Part model, mm, in its own coordinate system. A direction names the side the tool comes from. Coordinates: 2 decimals unless noted, no trailing zeros. Order: outer loops, then holes, each group sorted by start corner. A loop starts at its lowest first (then second) coordinate and runs counter-clockwise, first axis right, second up. Notation, with made-up numbers: (71, -18) - (104, -18) arc R22 cw to (104, 21) - close; hole circle Ø6 at (-31.5, -4). An arc over 180 degrees is marked (long way). Use a Markdown table: item, result. Add a question column.
1) Tool access for faces 5 (the face through (-19.86, 0.54, 14.84)), 6 (the face through (-13.25, 13.79, 3.06)), 7 (the face through (19.963, -13.457, -0.104)): list every direction of +Z, -Z, +X, -X, +Y, -Y with a clear straight run to the whole face (end or side of a thin tool).
2) Saw through at A-A on x = 11.5. List the corners of the cut face in (y, z), then the cut area to 3 significant figures.
3) Two-plate mould, pull along Z, no slides. Class faces 1 (the face through (21.151, -7.35, -7.35)), 2 (the face through (19.46, 15.62, 3.47)), 3 (the face through (21.82, 9.05, -4.71)), 4 (the face through (22.498, 12, -4)): +Z half, -Z half, draft (parallel to the pull), parting line (faces both ways), or undercut.
4) Wall check: L1, parallel to Y at x = -17.5, z = 0; L2, parallel to Y at x = 18, z = 0; L3, parallel to Z at x = 20.5, y = 0.5. Give the ranges that are in metal, low to high. Write a range as [from, to].
5) Drop flat-ended pins along their axis: P1, Ø4, axis at x = -1, y = -4.5, coming from the -Z side (3 decimals); P2, Ø1.4, axis at y = 0, z = -14.25, coming from the +X side; P3, Ø1.5, axis at y = -4.5, z = 6, coming from the +X side. Give the stop position or say it passes through.
```python
from build123d import *

# Parameters (mm, degrees)
HOLE_WIZARD_M2_1_D     = 1.6
HOLE_WIZARD_M2_1_DEPTH = 5
HOLE_WIZARD_M2_1_TIP   = 0.480688495
HOLE_WIZARD_M2_2_D     = 1.6
HOLE_WIZARD_M2_2_DEPTH = 5.2
HOLE_WIZARD_M2_2_TIP   = 0.480688495
SKETCH_9_R             = 1.25
CUT_EXTRUDE_1_DEPTH    = 20


with BuildPart() as part:
    # 草图1 → 旋转1 (revolve)
    with BuildSketch(Plane.XY, mode=Mode.PRIVATE) as revolve_1_sk:
        Polygon((16.5, 16), (13.035898385, 14), (-13.035898385, 14), (-16.5, 16), (-22.5, 16), (-22.5, 12.5), (17.00000944, 12.5), (17.004829984, 5.52730985), (18.592329605, 5.528407362), (22.501943889, 9.703811257), (22.501598217, 10.203809753), (21.151391042, 10.203809753), (21.151391042, 12.303809753), (22.497591042, 12.303809753), (22.497591042, 16), align=None)
    revolve(revolve_1_sk.sketch.rotate(Axis((22.5, 0, 0), (-1, 0, 0)), 90), axis=Axis((22.5, 0, 0), (-1, 0, 0)))

    # M2 螺纹孔1
    with Locations(Plane(origin=(22.497591042, 0, 0), x_dir=(0, 0, -1), z_dir=(1, 0, 0))):
        with Locations((0, 14.25), (14.25, 0), (0, -14.25), (-14.25, 0), (0, 0)):
            Hole(HOLE_WIZARD_M2_1_D / 2, depth=HOLE_WIZARD_M2_1_DEPTH)
            with Locations((0, 0, -(HOLE_WIZARD_M2_1_DEPTH + HOLE_WIZARD_M2_1_TIP / 2))):  # 118° drill point
                Cone(0, HOLE_WIZARD_M2_1_D / 2, HOLE_WIZARD_M2_1_TIP, mode=Mode.SUBTRACT)

    # M2 螺纹孔2
    with Locations(Plane.ZY.offset(22.5)):
        with Locations((0, 14.25), (14.25, 0), (0, -14.25), (-14.25, 0), (0, 0)):
            Hole(HOLE_WIZARD_M2_2_D / 2, depth=HOLE_WIZARD_M2_2_DEPTH)
            with Locations((0, 0, -(HOLE_WIZARD_M2_2_DEPTH + HOLE_WIZARD_M2_2_TIP / 2))):  # 118° drill point
                Cone(0, HOLE_WIZARD_M2_2_D / 2, HOLE_WIZARD_M2_2_TIP, mode=Mode.SUBTRACT)

    # 草图9 → 切除-拉伸1 (cut)
    with BuildSketch(Plane.XY):
        with Locations(Location((0, 0, 0), (0, 0, 180))):
            Circle(SKETCH_9_R)
    extrude(amount=CUT_EXTRUDE_1_DEPTH, mode=Mode.SUBTRACT)


solid = part.part
```
Results are:
| question | item | result |
|---|---|---|
| 1 | face 5 | -X |
| 1 | face 6 | none |
| 1 | face 7 | +X |
| 2 | outline | circle Ø28 at (0, 0); hole circle Ø25 at (0, 0) |
| 2 | area | 125 mm2 |
| 3 | face 1 | undercut |
| 3 | face 2 | parting line |
| 3 | face 3 | undercut |
| 3 | face 4 | draft |
| 4 | L1 | [-16, -15.05], [-13.45, -12.5], [12.5, 13.45], [15.05, 16] |
| 4 | L2 | [-16, -15.05], [-13.45, -5.53], [5.53, 13.45], [15.05, 16] |
| 4 | L3 | [-15.99, -14.87], [-13.63, -7.55], [7.55, 13.63], [14.87, 15.99] |
| 5 | P1 | z = -13.775 |
| 5 | P2 | x = 17.44 |
| 5 | P3 | x = 21.14 |
